Geometry check sheet. Reference: drawing and pictorial views, mm from the part's lowest x, y, z. Give positions to 0.01 mm unless a question says otherwise; leave off trailing zeros. Write each loop counter-clockwise with the first axis right and the second up, starting at its lowest first coordinate (ties: lowest second). Pieces come first, ordered by that corner, then holes. Notation, with made-up numbers: (11.5, 47.25) -> (63.5, 47.25) arc R14 cw to (63.5, 60.25) -> close; hole circle Ø5 at (34, 42). An arc over 180 degrees is marked (long way). Answer as CSV lines item,"result".
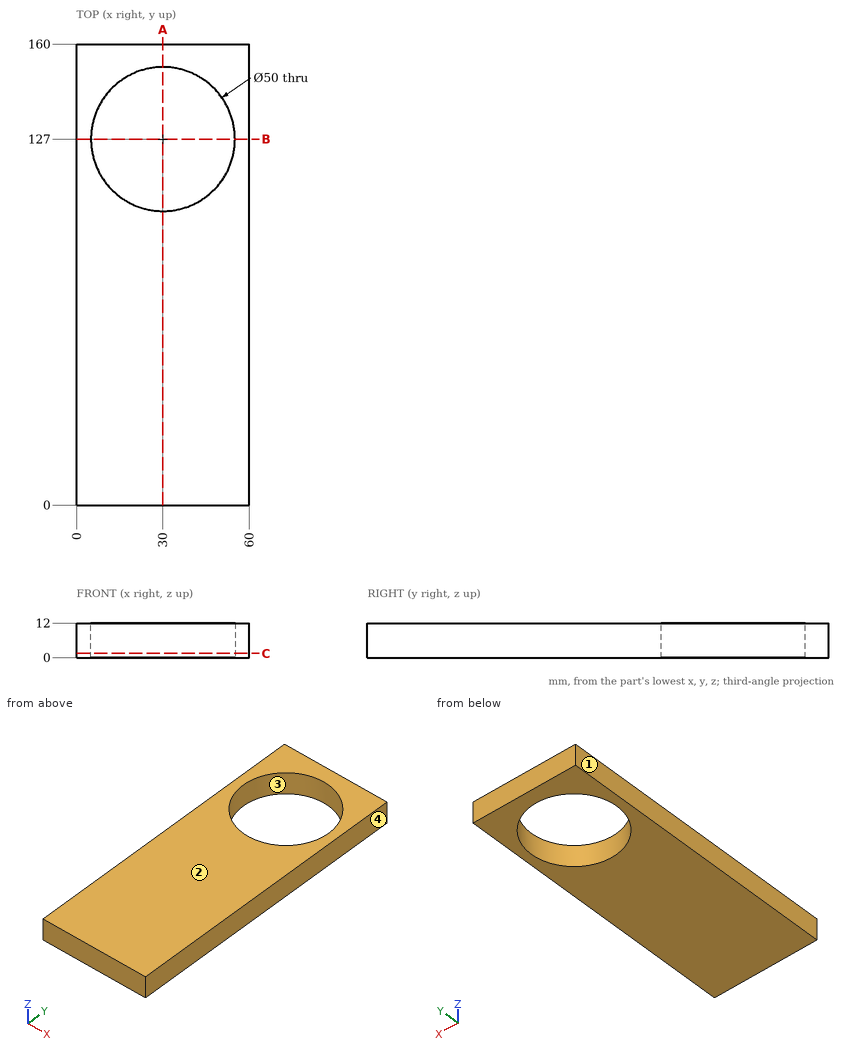
1) Depth check by flat-ended pin: pin 1 (4 mm diameter, centred on x = 51, z = 2, fed in from -Y). Enter the tip coordinate at first touch or a pass-through.
Reported:
pin 1,"y = 0"
2) Section check C-C (z = 1.5). Record the boundary of the cut face in (x, y).
Reported:
outline,"(0, 0) -> (60, 0) -> (60, 160) -> (0, 160) -> close; hole circle Ø50 at (30, 127)"
3) Section check A-A (x = 30). Record the boundary of the cut face in (y, z).
Reported:
outline,"(0, 0) -> (102, 0) -> (102, 12) -> (0, 12) -> close; (152, 0) -> (160, 0) -> (160, 12) -> (152, 12) -> close"
4) Scan lines: line 1 along Y through (x, z) = (30, 6.5); line 2 along X through (y, z) = (128, 8.5); line 3 along Y through (x, z) = (34, 10.5). Record each from-to range of solid material in increasing order.
Reported:
line 1,"0 to 102, 152 to 160"
line 2,"0 to 5.02, 54.98 to 60"
line 3,"0 to 102.32, 151.68 to 160"
5) Section check B-B (y = 127). Record the boundary of the cut face in (x, z), and give its area (3 significant figures).
Reported:
outline,"(0, 0) -> (5, 0) -> (5, 12) -> (0, 12) -> close; (55, 0) -> (60, 0) -> (60, 12) -> (55, 12) -> close"
area,"120 mm²"
6) Draft check along X on the marked faces 1, 2, 3 and 4. Enter one of: +X half, -X half, draft (parallel to the pull), parting line (faces both ways), or undercut.
Reported:
face 1,"-X half"
face 2,"draft"
face 3,"undercut"
face 4,"+X half"
